Check sheet for the drawn part. Datum: minimum x, y, z corner. Units: mm. A direction names the side the tool comes from. Give positions to 0.01 mm unless a question says otherwise; leave off trailing zeros. Write each loop counter-clockwise with the first axis right and the second up, starting at its lowest first coordinate (ties: lowest second). Pieces come first, ordered by that corner, then holes. Notation, with made-up numbers: (15.5, -14.5) - (23.5, -14.5) arc R35 cw to (23.5, 17.5) - close; hole circle Ø5 at (87, 63). An arc over 180 degrees is marked (long way). Answer as a JSON object with one key per item and string values. Group by question number.
Item 1: Draft check along Y on the marked faces 3, 4, 5 and 6. Enter one of: +Y half, -Y half, draft (parallel to the pull), parting line (faces both ways), or undercut.
Item 2: Sectioned sample at B-B, the plane y = 37.5. Record the boundary of the cut face in (x, z).
Item 3: Sectioned sample at A-A, the plane x = 229.5. Record the boundary of the cut face in (y, z).
Item 4: Go/stop test with flat-tipped pins: pin 1 (8 mm diameter, centred on y = 23, z = 38.5, fed in from +X); pin 2 (17 mm diameter, centred on x = 172, y = 19.5, fed in from -Z). Record where each tip stops, or that it passes through.
Item 5: Scan lines: line 1 along Z through (x, y) = (125.5, 40); line 2 along Y through (x, z) = (175, 3) (3 decimals). Record each from-to range of solid material in increasing order. Write a range as [from, to].
Item 6: Tool access check on the marked faces 1 and 2. Record the directions out of +Z, -Z, +X, -X, +Y, -Y that give a thin tool (end or side, any length) a straight path to the whole face; none if there is none.
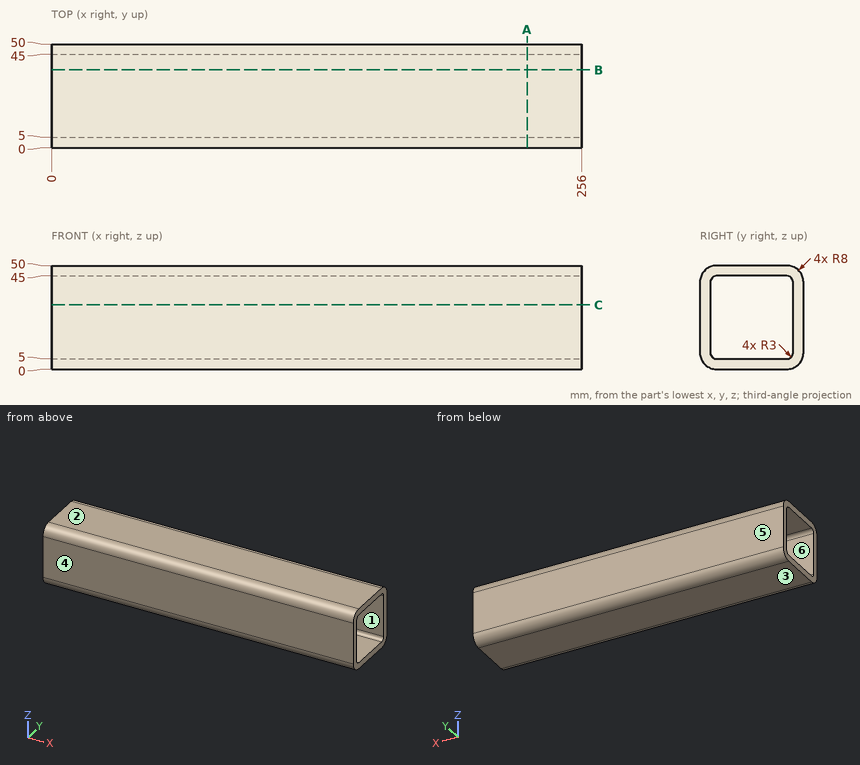
Geometry check:
{
 "1": {"face 3": "draft", "face 4": "-Y half", "face 5": "+Y half", "face 6": "undercut"},
 "2": {"outline": "(0, 0) - (256, 0) - (256, 5) - (0, 5) - close; (0, 45) - (256, 45) - (256, 50) - (0, 50) - close"},
 "3": {"outline": "(0, 8) arc R8 ccw to (8, 0) - (42, 0) arc R8 ccw to (50, 8) - (50, 42) arc R8 ccw to (42, 50) - (8, 50) arc R8 ccw to (0, 42) - close; hole (5, 8) arc R3 ccw to (8, 5) - (42, 5) arc R3 ccw to (45, 8) - (45, 42) arc R3 ccw to (42, 45) - (8, 45) arc R3 ccw to (5, 42) - close"},
 "4": {"pin 1": "through", "pin 2": "z = 0"},
 "5": {"line 1": "[0, 5], [45, 50]", "line 2": "[1.755, 48.245]"},
 "6": {"face 1": "+X, -X", "face 2": "+Z, +X, -X, +Y, -Y"}
}
